from build123d import *


with BuildPart() as part:
    # 草图1 → 旋转1 (revolve)
    with BuildSketch(Plane.XY):
        Polygon((7.5, 65.705286307), (0, 65.705286307), (0, 2.705286307), (15, 2.705286307), (15, 5.705286307), (12.5, 5.705286307), (12.5, 22.205286307), (11.5, 22.205286307), (11.5, 23.705286307), (12.5, 23.705286307), (12.5, 38.705286307), (10, 38.705286307), (10, 45.705286307), (7.5, 45.705286307), (7.5, 61.705286307), (6.7, 61.705286307), (6.7, 63.005286307), (7.5, 63.005286307), align=None)
    revolve(axis=Axis((0, 65.705286307, 0), (0, -1, 0)))


solid = part.part
Build history of the part. All positions in model axes, mm. A direction names the side the tool comes from. Coordinates: 2 decimals unless noted, no trailing zeros. Write each loop counter-clockwise with the first axis right and the second up, starting at its lowest first coordinate (ties: lowest second). Pieces come first, ordered by that corner, then holes.
(1) Mould opens along Y. For faces 4 (the flat face through (-0.1, 38.705, 10.2)), 5 (the cylindrical face through (-7.493, 53.817, 0.33)), 6 (the flat face through (-11, 23.705, -4)) say: pulls with the +Y half, pulls with the -Y half, needs draft (parallel to the pull), parting line crosses it, or undercut.
(2) Pin check, flat tips, straight feed: pin 1 Ø2 at (x, z) = (6.5, -8.5) entering from +Y; pin 2 Ø15 at (x, z) = (-2, -7.5) entering from +Y; pin 3 Ø8 at (x, y) = (-7, 13) entering from +Z; pin 4 Ø5 at (y, z) = (14, -12) entering from -X. Stop position of each tip, or through.
(3) Cut at C-C on y = 33.5. List the corners of the cut face in (x, z).
(4) Cut at D-D on x = 10.75. List the corners of the cut face in (y, z).
(5) 3-axis set-ups, long thin cutter, end or side, ignore diameter. For faces 1 (the flat face through (0, 2.705, 0)), 2 (the flat face through (0, 63.005, 7)), 3 (the cylindrical face through (-2.17, 42.25, -9.76)): which of +Z, -Z, +X, -X, +Y, -Y reach the whole face in a straight line?
(6) Drill centre lines: line 1 (Y direction, x = 1.75, z = 6.5); line 2 (Y direction, x = 12.5, z = -6.5); line 3 (Z direction, x = -0.25, y = 58.5). Where is each one in solid material? Low to high.
Working result:
1. face 4: pulls with the +Y half
1. face 5: needs draft
1. face 6: undercut
2. pin 1: stops at y = 45.71
2. pin 2: stops at y = 65.71
2. pin 3: stops at z = 12.13
2. pin 4: stops at x = -8.12
3. outline: circle Ø25 at (0, 0)
4. outline: (2.71, -10.46) - (5.71, -10.46) - (5.71, -6.38) - (22.21, -6.38) - (22.21, -4.09) - (23.71, -4.09) - (23.71, -6.38) - (38.71, -6.38) - (38.71, 6.38) - (23.71, 6.38) - (23.71, 4.09) - (22.21, 4.09) - (22.21, 6.38) - (5.71, 6.38) - (5.71, 10.46) - (2.71, 10.46) - close
5. face 1: +Z, -Z, +X, -X, -Y
5. face 2: none
5. face 3: +Y
6. line 1: y = 2.71 to 61.71, 63.01 to 65.71
6. line 2: y = 2.71 to 5.71
6. line 3: z = -7.5 to 7.5
